Model file for the job. Use its own axes, mm. Face numbers are marked on the shaded views. A direction names the side the tool comes from. Round coordinates to 2 decimals unless told otherwise and drop trailing zeros. Order: outer loops, then holes, each group sorted by start corner. A loop starts at its lowest first (then second) coordinate and runs counter-clockwise, first axis right, second up. Notation, with made-up numbers: (-18, 51) - (-9, 51) arc R19 ccw to (-9, 80) - close; hole circle Ø2 at (-21.5, 88.5). An arc over 180 degrees is marked (long way). Put each result on its own line as item: value. Start each with the question number.
Item 1: Which spindle directions (+Z, -Z, +X, -X, +Y, -Y) get a long thin tool onto all of the face, cutting with end or side? Do the marked faces 4 and 5. Say none if no direction does.
Item 2: Saw through at C-C on z = -14.5. List the corners of the cut face in (x, y), plus the area to 3 significant figures.
Item 3: Mould opens along Z. For the marked faces 1, 2 and 3 say: pulls with the +Z half, pulls with the -Z half, needs draft (parallel to the pull), parting line crosses it, or undercut.
Item 4: Saw through at B-B on y = -1. List the corners of the cut face in (x, z).
Item 5: Saw through at A-A on x = 0. List the corners of the cut face in (y, z).
Item 6: Saw through at D-D on z = -3.25. List the corners of the cut face in (x, y), plus the area to 3 significant figures.
Item 7: Pin check, flat tips, straight feed: pin 1 Ø8 at (y, z) = (3, -2) entering from +X; pin 2 Ø6 at (y, z) = (3, -5) entering from +X; pin 3 Ø1.5 at (x, y) = (6, 4) entering from +Z. Stop position of each tip, or through.
Item 8: Probe probe 1 along Z at (x, y) = (0, 3.75); probe 2 along Z at (x, y) = (5.5, -2.25); probe 3 along Z at (x, y) = (-5.5, -5.75). List the from-to ranges inside material, lowest first.
```python
from build123d import *


with BuildPart() as part:
    # Sketch1 → Revolve1 (revolve)
    with BuildSketch(Plane(origin=(0, 0, 0), x_dir=(0, 0, -1), z_dir=(1, 0, 0)), mode=Mode.PRIVATE) as revolve1_sk:
        Polygon((16.5, 0), (16.5, 8), (11.5, 8), (11.5, 6), (7, 6), (7, 3), (6, 3), (6, 4), (0, 4), (0, 0), align=None)
    revolve(revolve1_sk.sketch.rotate(Axis((0, 0, 0), (0, 0, -1)), 90), axis=Axis((0, 0, 0), (0, 0, -1)))


solid = part.part
```
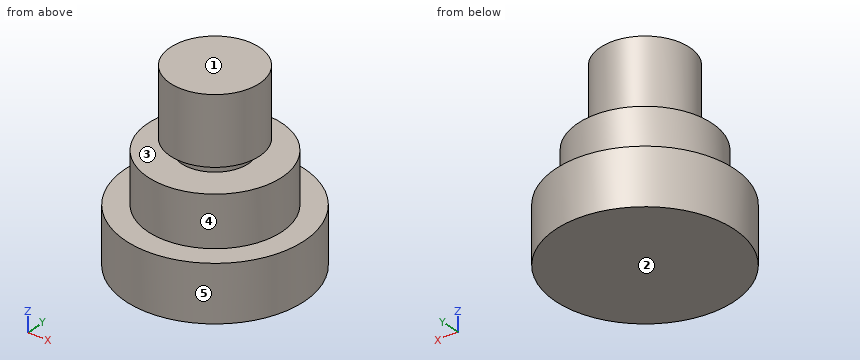
Results found:
1. face 4: +Z
1. face 5: +Z, -Z
2. outline: circle Ø16 at (0, 0)
2. area: 201 mm²
3. face 1: pulls with the +Z half
3. face 2: pulls with the -Z half
3. face 3: undercut
4. outline: (-7.94, -16.5) - (7.94, -16.5) - (7.94, -11.5) - (5.92, -11.5) - (5.92, -7) - (2.83, -7) - (2.83, -6) - (3.87, -6) - (3.87, 0) - (-3.87, 0) - (-3.87, -6) - (-2.83, -6) - (-2.83, -7) - (-5.92, -7) - (-5.92, -11.5) - (-7.94, -11.5) - close
5. outline: (-8, -16.5) - (8, -16.5) - (8, -11.5) - (6, -11.5) - (6, -7) - (3, -7) - (3, -6) - (4, -6) - (4, 0) - (-4, 0) - (-4, -6) - (-3, -6) - (-3, -7) - (-6, -7) - (-6, -11.5) - (-8, -11.5) - close
6. outline: circle Ø8 at (0, 0)
6. area: 50.3 mm²
7. pin 1: stops at x = 4
7. pin 2: stops at x = 5.95
7. pin 3: stops at z = -11.5
8. probe 1: z = -16.5 to -7, -6 to 0
8. probe 2: z = -16.5 to -7
8. probe 3: z = -16.5 to -11.5
